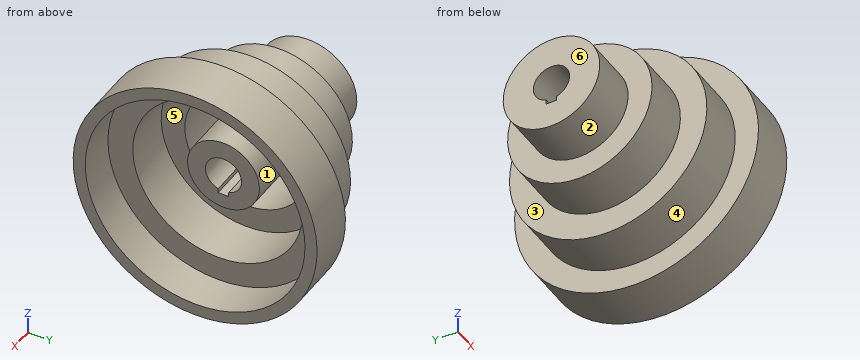
from build123d import *

# Parameters (mm, degrees)
BORE_AND_KEYWAY_PROFILE_W    = 15
BORE_AND_KEYWAY_PROFILE_H    = 8.680150088
SHAFT_BORE_WITH_KEYWAY_DEPTH = 110


with BuildPart() as part:
    # Stepped Pulley Profile → Stepped Pulley Body (revolve)
    with BuildSketch(Plane.XY, mode=Mode.PRIVATE) as stepped_pulley_body_sk:
        Polygon((-55.070008805, 15), (-55.070008805, 40), (-15.070008805, 40), (-15.070008805, 59.802619068), (24.929991195, 59.802619068), (24.929991195, 81.746061819), (64.929991195, 81.746061819), (64.929991195, 101.013474967), (104.929991195, 101.013474967), (104.929991195, 91.013474967), (72.929991195, 91.013474967), (72.929991195, 70.393812799), (32.929991195, 70.393812799), (32.929991195, 50.858796691), (-7.070008805, 50.858796691), (-7.070008805, 29.765145873), (64.929991195, 29.765145873), (64.929991195, 15), align=None)
    revolve(stepped_pulley_body_sk.sketch.rotate(Axis((151.689826596, 0, 0), (-1, 0, 0)), 90), axis=Axis((151.689826596, 0, 0), (-1, 0, 0)))

    # Bore and Keyway Profile → Shaft Bore with Keyway (cut, symmetric)
    with BuildSketch(Plane(origin=(0, 0, 0), x_dir=(0, 0, -1), z_dir=(1, 0, 0))):
        with Locations((10.5, 0)):
            Rectangle(BORE_AND_KEYWAY_PROFILE_W, BORE_AND_KEYWAY_PROFILE_H)
    extrude(amount=SHAFT_BORE_WITH_KEYWAY_DEPTH, both=True, mode=Mode.SUBTRACT)


solid = part.part
The listing builds one solid part. Answer for the finished solid, in the listing's coordinates (mm). Face numbers are marked on the shaded views. A direction names the side the tool comes from. Give positions to 0.01 mm unless a question says otherwise; leave off trailing zeros. Write each loop counter-clockwise with the first axis right and the second up, starting at its lowest first coordinate (ties: lowest second). Pieces come first, ordered by that corner, then holes.
1) Section A-A (x = -4) is taken. Write down the section's boundary in (y, z), and give its area (3 significant figures).
2) Given P1, Ø1.5, axis at y = 47.5, z = -32, coming from the +X side; P2, Ø12, axis at x = -13.5, z = 8, coming from the -Y side; P3, Ø1.8, axis at x = 28, z = -15.5, coming from the +Y side, each flat-ended and moving along its own axis, determine where each tip first touches the part or whether it passes through.
3) A tool of negligible diameter and unlimited length cuts with its end or side. For the marked faces 4, 5 and 6, from which of +Z, -Z, +X, -X, +Y, -Y can it reach the whole face along a straight path? Write none if from no direction.
4) Section B-B (x = -23.5) is taken. Write down the section's boundary in (y, z), and give its area (3 significant figures).
5) Find the intervals of material crossed by L1, parallel to Y at x = 12, z = 0; L2, parallel to Y at x = 61, z = 0; L3, parallel to Y at x = 98, z = 0, in increasing order.
6) Section D-D (z = 86) is taken. Write down the section's boundary in (x, y).
7) For a pull along Z with two mould halves and no side action, classify the marked faces 1, 2 and 3 as pulls with the +Z half, pulls with the -Z half, needs draft (parallel to the pull), parting line crosses it, or undercut.
Response:
1. outline: circle Ø119.61 at (0, 0); circle Ø59.53 at (0, 0); hole circle Ø101.72 at (0, 0); hole (-4.34, -18) - (4.34, -18) - (4.34, -14.36) arc R15 ccw (long way) to (-4.34, -14.36) - close
1. area: 5,160 mm2
2. P1: stops at x = 32.93
2. P2: stops at y = -59.77
2. P3: stops at y = 80.43
3. face 4: -X
3. face 5: +X
3. face 6: +Z, -Z, -X, +Y, -Y
4. outline: circle Ø80 at (0, 0); hole (-4.34, -18) - (4.34, -18) - (4.34, -14.36) arc R15 ccw (long way) to (-4.34, -14.36) - close
4. area: 4,290 mm2
5. L1: y = -59.8 to -50.86, -29.77 to -15, 15 to 29.77, 50.86 to 59.8
5. L2: y = -81.75 to -70.39, -29.77 to -15, 15 to 29.77, 70.39 to 81.75
5. L3: y = -101.01 to -91.01, 91.01 to 101.01
6. outline: (64.93, -52.99) - (104.93, -52.99) - (104.93, -29.79) - (72.93, -29.79) - (72.93, 29.79) - (104.93, 29.79) - (104.93, 52.99) - (64.93, 52.99) - close
7. face 1: undercut
7. face 2: parting line crosses it
7. face 3: needs draft
